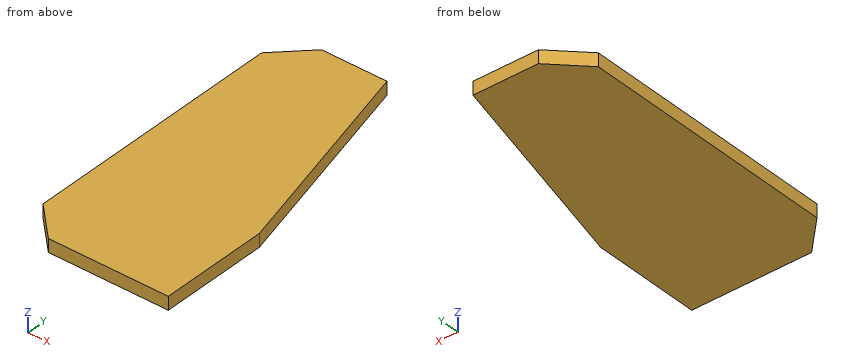
from build123d import *

# Parameters (mm, degrees)
BOSS_EXTRUDE1_DEPTH = 6
CHAMFER1_SIZE       = 15


with BuildPart() as part:
    # Sketch1 → Boss-Extrude1 (new body)
    with BuildSketch(Plane.XY):
        Polygon((0, 150), (0, 0), (70, 0), (70, 50), (45, 150), align=None)
    extrude(amount=BOSS_EXTRUDE1_DEPTH)

    # Chamfer1
    chamfer1_edges = [part.edges().sort_by_distance(p)[0] for p in [
        (0, 0, 3),
        (0, 150, 3),
    ]]
    chamfer(chamfer1_edges, length=CHAMFER1_SIZE)


solid = part.part
Geometry: final body of the model. Coordinates: model frame, mm. Give positions to 0.01 mm unless a question says otherwise; leave off trailing zeros. Write each loop counter-clockwise with the first axis right and the second up, starting at its lowest first coordinate (ties: lowest second). Pieces come first, ordered by that corner, then holes. Notation, with made-up numbers: M -39.75,53 L 15.25,53 A24 cw 15.25,83 Z; hole C -32,18.5 d3. An arc over 180 degrees is marked long. Answer in a Markdown table with one row per item. Add a question column.
(1) Ray query, line 1 (X direction, y = 75, z = 2.5); line 2 (X direction, y = 52.5, z = 1.25) (3 decimals); line 3 (Y direction, x = 6.5, z = 1.6). Return the intervals inside material, ascending.
(2) Section B-B on x = 61. Return loops of the section in (y, z).
(3) First-contact query: pin 1 (3 mm diameter, centred on x = 12, z = 1, fed in from -Y). Flat tip, straight axial feed; report the tip coordinate or a pass-through.
(4) Section A-A on z = 4.9. Return loops of the section in (x, y), and give its area (4 significant figures).
(5) Section C-C on y = 139. Return loops of the section in (x, z).
Result set:
| question | item | result |
|---|---|---|
| 1 | line 1 | x = 0 to 63.75 |
| 1 | line 2 | x = 0 to 69.375 |
| 1 | line 3 | y = 8.5 to 141.5 |
| 2 | outline | M 0,0 L 86,0 L 86,6 L 0,6 Z |
| 3 | pin 1 | stops at y = 1.5 |
| 4 | outline | M 0,15 L 15,0 L 70,0 L 70,50 L 45,150 L 15,150 L 0,135 Z |
| 4 | area | 9,025 mm^2 |
| 5 | outline | M 4,0 L 47.75,0 L 47.75,6 L 4,6 Z |
